For this review, take the finished solid that the model builds, in its own axes (mm). Face numbers are marked on the shaded views. A direction names the side the tool comes from. Give positions to 0.01 mm unless a question says otherwise; leave off trailing zeros. Loops run counter-clockwise (first coordinate to the right, second up) from the corner with the lowest first, then second, coordinate; pieces in that order, holes last.
```python
from build123d import *

# Parameters (mm, degrees)
SKETCH1_R           = 28
BOSS_EXTRUDE1_DEPTH = 13
SKETCH2_R           = 25
BOSS_EXTRUDE2_DEPTH = 3
CHAMFER1_SIZE       = 1


with BuildPart() as part:
    # Sketch1 → Boss-Extrude1 (new body)
    with BuildSketch(Plane.XY):
        with Locations(Location((0, 0, 0), (0, 0, 180))):
            Circle(SKETCH1_R)
    extrude(amount=BOSS_EXTRUDE1_DEPTH)

    # Sketch2 → Boss-Extrude2 (add)
    with BuildSketch(Plane.XY.offset(13)):
        Circle(SKETCH2_R)
    extrude(amount=BOSS_EXTRUDE2_DEPTH)

    # Chamfer1
    chamfer1_edges = [part.edges().sort_by_distance(p)[0] for p in [
        (28, 0, 0),
        (-25, 0, 16),
    ]]
    chamfer(chamfer1_edges, length=CHAMFER1_SIZE)

    # Sketch4 → G1-1/4 Tapped Hole1 (revolve, cut)
    with BuildSketch(Plane(origin=(0, 0, 16), x_dir=(0, -1, 0), z_dir=(1, 0, 0))):
        Polygon((0, 0), (0, 102.538889648), (19.625, 90.747), (19.625, 0), align=None)
    revolve(axis=Axis((0, 0, 22.35), (0, 0, -1)), mode=Mode.SUBTRACT)


solid = part.part
```
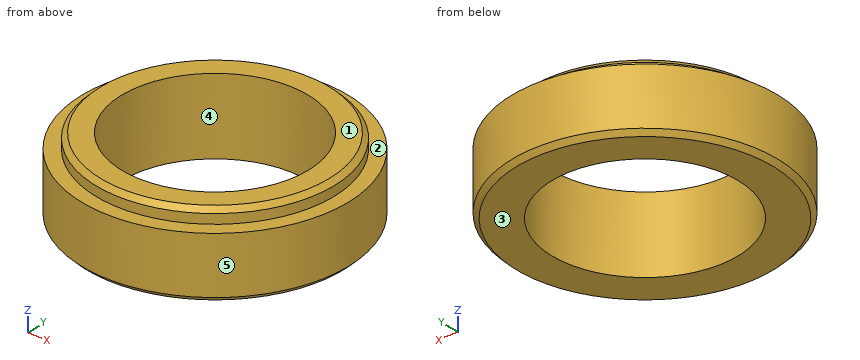
Q1. For pin 1 Ø1 at (y, z) = (-19.5, 3) entering from +X; pin 2 Ø8 at (x, z) = (19.5, 14) entering from +Y; pin 3 Ø17 at (x, y) = (8, 7) entering from +Z; pin 4 Ø3 at (x, y) = (-21, 14) entering from +Z, all flat-tipped, find the tip position at first contact; note any pin that passes through.
Answers:
pin 1: stops at x = 20.57
pin 2: stops at y = 23.23
pin 3: passes through
pin 4: stops at z = 16
Q2. Machinability: for the marked faces 1 and 2, which of the approach directions +Z, -Z, +X, -X, +Y, -Y give a long, thin tool a straight path to every point of the face, cutting with its end or side? Answer none if there is none.
Answers:
face 1: +Z, +X, -X, +Y, -Y
face 2: +Z
Q3. For probe 1 along Y at (x, z) = (0, 6.25) (3 decimals); probe 2 along Y at (x, z) = (4.5, 4); probe 3 along X at (y, z) = (9.5, 12.25), list the stretches that pass through material, from the lowest coordinate up.
Answers:
probe 1: y = -28 to -19.625, 19.625 to 28
probe 2: y = -27.64 to -19.1, 19.1 to 27.64
probe 3: x = -26.34 to -17.17, 17.17 to 26.34
Q4. Mouldability with a two-part tool opening along Y and no side actions: class the marked faces 3, 4 and 5 as +Y half, -Y half, draft (parallel to the pull), parting line (faces both ways), or undercut.
Answers:
face 3: draft
face 4: undercut
face 5: parting line
Q5. Consider section C-C on z = 7.75. Give the boundary of the cut face in (x, y) (3 decimals), plus the area to 3 significant figures.
Answers:
outline: circle Ø56 at (0, 0); hole circle Ø39.25 at (0, 0)
area: 1,250 mm2
Q6. Consider section A-A on y = 0. Give the boundary of the cut face in (x, z) (3 decimals), plus the area to 3 significant figures.
Answers:
outline: (-28, 1) - (-27, 0) - (-19.625, 0) - (-19.625, 16) - (-24, 16) - (-25, 15) - (-25, 13) - (-28, 13) - close; (19.625, 0) - (27, 0) - (28, 1) - (28, 13) - (25, 13) - (25, 15) - (24, 16) - (19.625, 16) - close
area: 248 mm2
